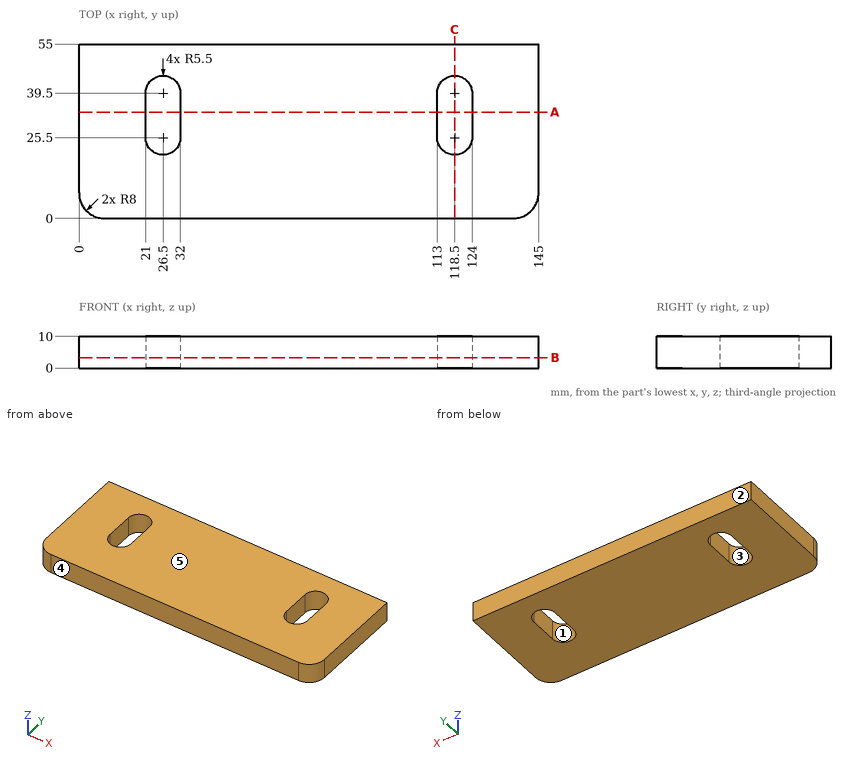
Can you work these out from the drawing? Everything is in mm from the part's minimum corner. A direction names the side the tool comes from. Round coordinates to 2 decimals unless told otherwise and drop trailing zeros. Write each loop counter-clockwise with the first axis right and the second up, starting at its lowest first coordinate (ties: lowest second). Pieces come first, ordered by that corner, then holes. Notation, with made-up numbers: (-13, 83) - (1, 83) arc R7 ccw to (1, 95) - close; hole circle Ø3 at (-34, -5). An arc over 180 degrees is marked (long way). Use a Markdown table: item, result.
Q1. For pin 1 (12 mm diameter, centred on x = 114.5, y = 29.5, fed in from -Z), with a flat end and sliding along its axis, tell me the tip position at first contact or that it passes through.
Output values:
| item | result |
|---|---|
| pin 1 | z = 0 |
Q2. I want a section at A-A (y = 33.5). List the corners of the cut face in (x, z) for me, plus the area to 3 significant figures.
Output values:
| item | result |
|---|---|
| outline | (0, 0) - (21, 0) - (21, 10) - (0, 10) - close; (32, 0) - (113, 0) - (113, 10) - (32, 10) - close; (124, 0) - (145, 0) - (145, 10) - (124, 10) - close |
| area | 1,230 mm2 |
Q3. Thinking about a two-plate mould opening in Y: for the marked faces 3, 4 and 5, which applies, released by +Y, released by -Y, zero draft, split by the parting line, or undercut?
Output values:
| item | result |
|---|---|
| face 3 | undercut |
| face 4 | released by -Y |
| face 5 | zero draft |
Q4. I want a section at B-B (z = 3.25). List the corners of the cut face in (x, y) for me, plus the area to 3 significant figures.
Output values:
| item | result |
|---|---|
| outline | (0, 8) arc R8 ccw to (8, 0) - (137, 0) arc R8 ccw to (145, 8) - (145, 55) - (0, 55) - close; hole (21, 25.5) arc R5.5 ccw to (32, 25.5) - (32, 39.5) arc R5.5 ccw to (21, 39.5) - close; hole (113, 25.5) arc R5.5 ccw to (124, 25.5) - (124, 39.5) arc R5.5 ccw to (113, 39.5) - close |
| area | 7,450 mm2 |
Q5. Please list where these lines run through material, in increasing order: L1, parallel to X at y = 34, z = 6.5; L2, parallel to X at y = 42.5, z = 6; L3, parallel to Y at x = 29.5, z = 1.
Output values:
| item | result |
|---|---|
| L1 | 0 to 21, 32 to 113, 124 to 145 |
| L2 | 0 to 21.89, 31.11 to 113.89, 123.11 to 145 |
| L3 | 0 to 20.89, 44.11 to 55 |
Q6. For the marked faces 1 and 2, which set-ups out of +Z, -Z, +X, -X, +Y, -Y let a thin tool reach every point of the face, with its end or its side?
Output values:
| item | result |
|---|---|
| face 1 | +Z, -Z |
| face 2 | +Z, -Z, +X, -X, +Y |
Q7. I want a section at C-C (x = 118.5). List the corners of the cut face in (y, z) for me.
Output values:
| item | result |
|---|---|
| outline | (0, 0) - (20, 0) - (20, 10) - (0, 10) - close; (45, 0) - (55, 0) - (55, 10) - (45, 10) - close |
